```python
from build123d import *

# Parameters (mm, degrees)
SWEEP_1_PROFILE_R   = 13.5
SWEEP_1_PROFILE_R_2 = 12.5


with BuildPart() as part:
    # 扫描-薄件1: sweep along a path in 草图1
    with BuildLine(Plane.XY) as sweep_1_path:
        Line((-575, 0), (-575, 450))
        ThreePointArc((-575, 450), (-545.710678119, 520.710678119), (-475, 550))
        Line((-475, 550), (475, 550))
        ThreePointArc((475, 550), (545.710678119, 520.710678119), (575, 450))
        Line((575, 450), (575, 0))
    # 扫描-薄件1 profile (on start of the path) → 扫描-薄件1 (sweep)
    with BuildSketch(Plane(origin=(-575, 0, 0), x_dir=(0, 0, 1), z_dir=(0, 1, 0))):
        Circle(SWEEP_1_PROFILE_R)
        Circle(SWEEP_1_PROFILE_R_2, mode=Mode.SUBTRACT)
    sweep(path=sweep_1_path.line)


solid = part.part
```
Geometry: final body of the model. Coordinates: model frame, mm. A direction names the side the tool comes from. Coordinates: 2 decimals unless noted, no trailing zeros. Order: outer loops, then holes, each group sorted by start corner. A loop starts at its lowest first (then second) coordinate and runs counter-clockwise, first axis right, second up. Notation, with made-up numbers: (68, -8.75) - (84, -8.75) arc R28 ccw to (84, 20.25) - close; hole circle Ø7 at (15, 65.5). An arc over 180 degrees is marked (long way). Return JSON: item names as keys, results as strings. Group by question number.
1. Cut plane B-B (y = 397). Output: boundary loops of the cut face in (x, z), plus the area to 3 significant figures.
2. Pull-direction query (Y, two-part tool) for faces 1 (the face through (-584, 0, 9)), 2 (the face through (587.203, 221.85, -2.71)), 3 (the face through (6.65, 536.615, -1.757)), 4 (the face through (6.65, 562.203, -2.71)); classes: pulls with the +Y half, pulls with the -Y half, needs draft (parallel to the pull), parting line crosses it, or undercut.
3. Pin query (flat end, axial travel): pin 1 (10 mm diameter, centred on y = 177, z = 7.5, fed in from +X); pin 2 (2 mm diameter, centred on y = 148, z = -10, fed in from +X); pin 3 (1 mm diameter, centred on y = 361, z = -5.5, fed in from +X). Return the tip coordinate at first contact, or that it passes through.
4. Cut plane C-C (x = 40). Output: boundary loops of the cut face in (y, z), plus the area to 3 significant figures.
5. Set-up query: faces 5 (the face through (-561.615, 228.15, -1.757)), 6 (the face through (566, 0, -9)). Return all of +Z, -Z, +X, -X, +Y, -Y with unobstructed straight access to the full face (end or side cutting, diameter ignored); none if empty.
6. Cut plane A-A (z = 0). Output: boundary loops of the cut face in (x, y), plus the area to 3 significant figures.
7. Material intervals for line 1 along X through (y, z) = (302.5, 0); line 2 along X through (y, z) = (330, -1.25); line 3 along Z through (x, y) = (-152, 550), sorted ascending. Write a range as [from, to].
8. Cut plane D-D (y = 462). Count the separate pieces of the cut face and the enclosed holes in it, plus the area to 3 significant figures.
Resolved:
{
 "1": {"outline": "circle Ø27 at (-575, 0); circle Ø27 at (575, 0); hole circle Ø25 at (-575, 0); hole circle Ø25 at (575, 0)", "area": "163 mm²"},
 "2": {"face 1": "pulls with the -Y half", "face 2": "needs draft", "face 3": "parting line crosses it", "face 4": "undercut"},
 "3": {"pin 1": "stops at x = 588.27", "pin 2": "stops at x = 585.06", "pin 3": "stops at x = 587.54"},
 "4": {"outline": "circle Ø27 at (550, 0); hole circle Ø25 at (550, 0)", "area": "81.7 mm²"},
 "5": {"face 5": "-Y", "face 6": "+Z, -Z, +X, -X, -Y"},
 "6": {"outline": "(-588.5, 0) - (-587.5, 0) - (-587.5, 450) arc R112.5 cw to (-475, 562.5) - (475, 562.5) arc R112.5 cw to (587.5, 450) - (587.5, 0) - (588.5, 0) - (588.5, 450) arc R113.5 ccw to (475, 563.5) - (-475, 563.5) arc R113.5 ccw to (-588.5, 450) - close; (-562.5, 0) - (-561.5, 0) - (-561.5, 450) arc R86.5 cw to (-475, 536.5) - (475, 536.5) arc R86.5 cw to (561.5, 450) - (561.5, 0) - (562.5, 0) - (562.5, 450) arc R87.5 ccw to (475, 537.5) - (-475, 537.5) arc R87.5 ccw to (-562.5, 450) - close", "area": "4,330 mm²"},
 "7": {"line 1": "x = [-588.5, -587.5], [-562.5, -561.5], [561.5, 562.5], [587.5, 588.5]", "line 2": "x = [-588.44, -587.44], [-562.56, -561.56], [561.56, 562.56], [587.44, 588.44]", "line 3": "z = [-13.5, -12.5], [12.5, 13.5]"},
 "8": {"separate pieces": "2", "enclosed holes": "2", "area": "165 mm²"}
}
